The model under review builds one solid part; all positions refer to its coordinate system, in mm. A direction names the side the tool comes from. Give positions to 0.01 mm unless a question says otherwise; leave off trailing zeros. Loops run counter-clockwise (first coordinate to the right, second up) from the corner with the lowest first, then second, coordinate; pieces in that order, holes last. Notation, with made-up numbers: M 73.25,1.25 L 124.25,1.25 A31 cw 124.25,38.25 Z; hole C 77.5,-15.75 d4. An arc over 180 degrees is marked long. Write item = value, one per line. Start each with the question number.
1. We need section C-C on z = -22. Give the boundary of the cut face in (x, y).
2. We need section D-D on y = 186. Give the boundary of the cut face in (x, z).
3. We need section B-B on x = -142.25. Give the boundary of the cut face in (y, z).
4. For faces 1 (the face through (-149.42, 179.15, -8)), 2 (the face through (-143.35, 177.2, -28.26)), 3 (the face through (-146, 181, -46)), list the 3-axis set-ups (+Z, -Z, +X, -X, +Y, -Y) from which the entire face can be reached by the end or side of a thin tool; tool diameter is ignored.
5. We need section A-A on y = 177.5. Give the boundary of the cut face in (x, z).
6. For pin 1 (2 mm diameter, centred on x = -149, z = -9, fed in from -Y); pin 2 (6 mm diameter, centred on y = 185, z = -10, fed in from +X); pin 3 (5 mm diameter, centred on x = -143, z = -23, fed in from -Y), all flat-tipped, find the tip position at first contact; note any pin that passes through.
7. Wall thickness on line 1 along Z through (x, y) = (-140.5, 179.25); line 2 along Y through (x, z) = (-145.5, -31); line 3 along Y through (x, z) = (-148.25, -34): over which ranges is each line inside the solid? List them lowest first. Write a range as from..to.
from build123d import *

# Parameters (mm, degrees)
SKETCH_1_R      = 4
EXTRUDE_1_DEPTH = 8
SKETCH_2_R      = 6
EXTRUDE_2_DEPTH = 3
SKETCH_3_R      = 4
EXTRUDE_3_DEPTH = 30
SKETCH_4_R      = 4
EXTRUDE_4_DEPTH = 5


with BuildPart() as part:
    # 草图1 → 凸台-拉伸1 (new body)
    with BuildSketch(Plane.XY):
        with Locations((-145.504664302, 180.568940096)):
            Circle(SKETCH_1_R)
    extrude(amount=-EXTRUDE_1_DEPTH)

    # 草图2 → 凸台-拉伸2 (add)
    with BuildSketch(Plane(origin=(0, 0, -8), x_dir=(-1, 0, 0), z_dir=(0, 0, -1))):
        with Locations(Location((145.504664302, 180.568940096, 0), (0, 0, 90))):
            Circle(SKETCH_2_R)
    extrude(amount=EXTRUDE_2_DEPTH)

    # 草图3 → 凸台-拉伸3 (add)
    with BuildSketch(Plane(origin=(0, 0, -11), x_dir=(-1, 0, 0), z_dir=(0, 0, -1))):
        with Locations(Location((145.504664302, 180.568940096, 0), (0, 0, 180))):
            Circle(SKETCH_3_R)
    extrude(amount=EXTRUDE_3_DEPTH)

    # 草图4 → 凸台-拉伸4 (add)
    with BuildSketch(Plane(origin=(0, 0, -41), x_dir=(-1, 0, 0), z_dir=(0, 0, -1))):
        with Locations(Location((145.504664302, 180.568940096, 0), (0, 0, 180))):
            Circle(SKETCH_4_R)
    extrude(amount=EXTRUDE_4_DEPTH)


solid = part.part
Final values:
q1.outline = C -145.5,180.57 d8
q2.outline = M -148.05,-11 L -142.95,-11 L -142.95,-8 L -148.05,-8 Z
q3.outline = M 175.53,-11 L 178.24,-11 L 178.24,-46 L 182.89,-46 L 182.89,-11 L 185.61,-11 L 185.61,-8 L 182.89,-8 L 182.89,0 L 178.24,0 L 178.24,-8 L 175.53,-8 Z
q4.face_1 = +Z
q4.face_2 = -Z
q4.face_3 = -Z, +X, -X, +Y, -Y
q5.outline = M -150.66,-11 L -148.07,-11 L -148.07,-46 L -142.94,-46 L -142.94,-11 L -140.35,-11 L -140.35,-8 L -142.94,-8 L -142.94,0 L -148.07,0 L -148.07,-8 L -150.66,-8 Z
q6.pin_1 = 175.11
q6.pin_2 = -139.68
q6.pin_3 = 176.57
q7.line_1 = -11..-8
q7.line_2 = 176.57..184.57
q7.line_3 = 177.66..183.48
